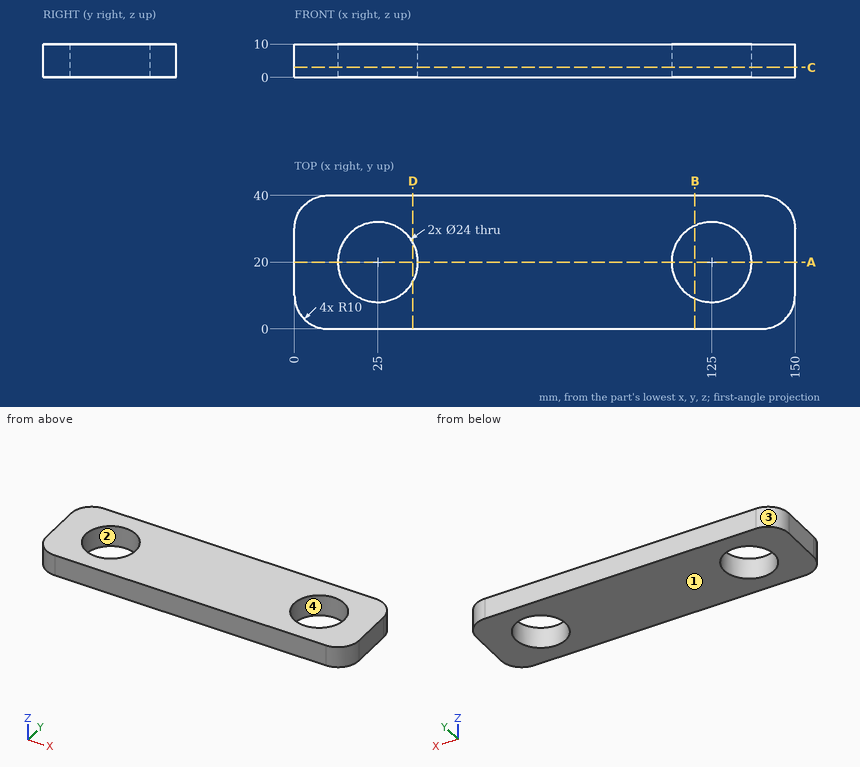
Answer from the drawing. Dimensions are ordinates in mm from the lowest x, y and z of the part. Round coordinates to 2 decimals unless told otherwise and drop trailing zeros. Write each loop counter-clockwise with the first axis right and the second up, starting at its lowest first coordinate (ties: lowest second). Pieces come first, ordered by that corner, then holes.
1. The part is cut by section B-B, the plane x = 120. Determine the outline of the cut face in (y, z).
2. The part is cut by section C-C, the plane z = 3. Determine the outline of the cut face in (x, y), then the cut area to 3 significant figures.
3. The part is cut by section A-A, the plane y = 20. Determine the outline of the cut face in (x, z).
4. The part is cut by section D-D, the plane x = 35.5. Determine the outline of the cut face in (y, z).
5. Given pin 1 Ø14.5 at (x, y) = (25, 20) entering from +Z; pin 2 Ø1.5 at (x, z) = (115, 6.5) entering from -Y, each flat-ended and moving along its own axis, determine where each tip first touches the part or whether it passes through.
6. Straight lines are drawn through the part: L1, parallel to Y at x = 25, z = 1.5; L2, parallel to X at y = 28, z = 6.75; L3, parallel to X at y = 22, z = 5.25. For each, find the intervals that lie inside material, in ascending order.
7. Determine the mould class of the marked faces 1, 2, 3 and 4 for opening direction Y: pulls with the +Y half, pulls with the -Y half, needs draft (parallel to the pull), parting line crosses it, or undercut.
Values:
1. outline: (0, 0) - (9.09, 0) - (9.09, 10) - (0, 10) - close; (30.91, 0) - (40, 0) - (40, 10) - (30.91, 10) - close
2. outline: (0, 10) arc R10 ccw to (10, 0) - (140, 0) arc R10 ccw to (150, 10) - (150, 30) arc R10 ccw to (140, 40) - (10, 40) arc R10 ccw to (0, 30) - close; hole circle Ø24 at (25, 20); hole circle Ø24 at (125, 20)
2. area: 5,010 mm2
3. outline: (0, 0) - (13, 0) - (13, 10) - (0, 10) - close; (37, 0) - (113, 0) - (113, 10) - (37, 10) - close; (137, 0) - (150, 0) - (150, 10) - (137, 10) - close
4. outline: (0, 0) - (14.19, 0) - (14.19, 10) - (0, 10) - close; (25.81, 0) - (40, 0) - (40, 10) - (25.81, 10) - close
5. pin 1: passes through
5. pin 2: stops at y = 0
6. L1: y = 0 to 8, 32 to 40
6. L2: x = 0 to 16.06, 33.94 to 116.06, 133.94 to 150
6. L3: x = 0 to 13.17, 36.83 to 113.17, 136.83 to 150
7. face 1: needs draft
7. face 2: undercut
7. face 3: pulls with the +Y half
7. face 4: undercut
